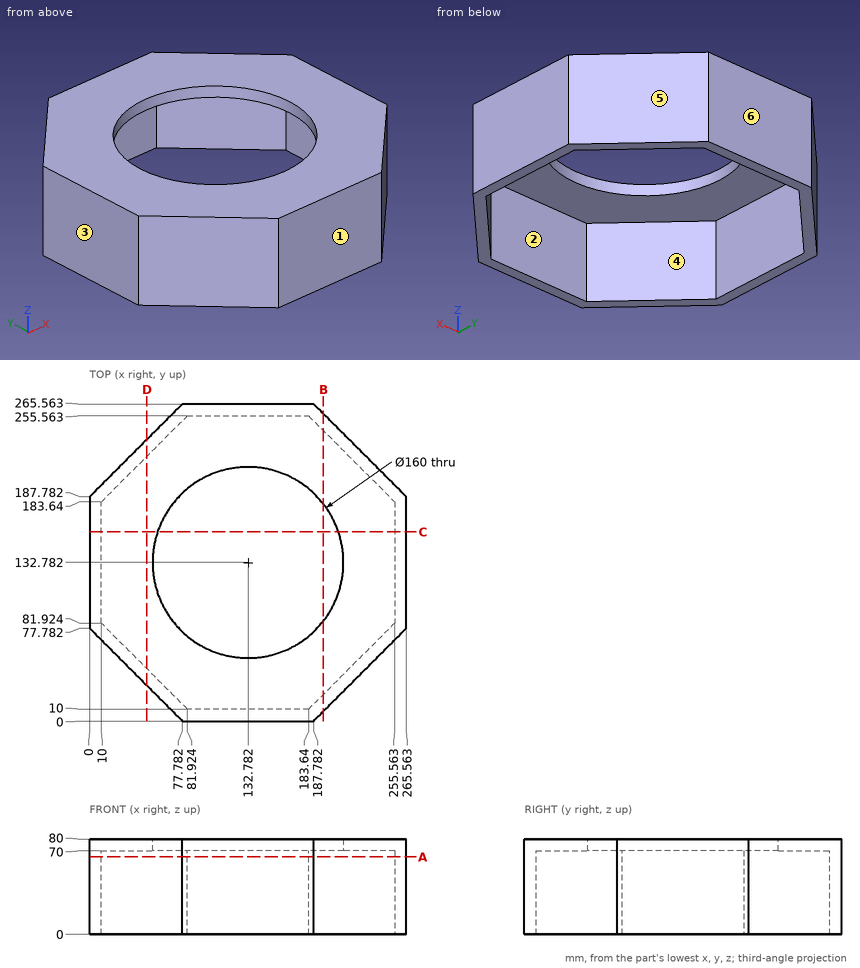
Can you work these out from the drawing? Everything is in mm from the part's minimum corner. A direction names the side the tool comes from. Round coordinates to 2 decimals unless told otherwise and drop trailing zeros. Order: outer loops, then holes, each group sorted by start corner. A loop starts at its lowest first (then second) coordinate and runs counter-clockwise, first axis right, second up. Notation, with made-up numbers: (-27.75, 16.5) - (-18.75, 16.5) arc R9 cw to (-18.75, 23.5) - close; hole circle Ø5 at (3, 31). An arc over 180 degrees is marked (long way). Answer in a Markdown table with one row per item.
(1) Suppose I cut it at A-A, the plane z = 65. Please give me the cut outline in (x, y).
From the geometry:
| item | result |
|---|---|
| outline | (0, 77.78) - (77.78, 0) - (187.78, 0) - (265.56, 77.78) - (265.56, 187.78) - (187.78, 265.56) - (77.78, 265.56) - (0, 187.78) - close; hole (10, 81.92) - (81.92, 10) - (183.64, 10) - (255.56, 81.92) - (255.56, 183.64) - (183.64, 255.56) - (81.92, 255.56) - (10, 183.64) - close |
(2) Suppose I cut it at C-C, the plane y = 158.5. Please give me the cut outline in (x, z) (1 decimal).
From the geometry:
| item | result |
|---|---|
| outline | (0, 0) - (10, 0) - (10, 70) - (57, 70) - (57, 80) - (0, 80) - close; (208.5, 70) - (255.6, 70) - (255.6, 0) - (265.6, 0) - (265.6, 80) - (208.5, 80) - close |
(3) If we mould it in two halves opening along X, with no side actions, what happens to the marked faces 3, 4, 5 and 6? For each: released by +X, released by -X, zero draft, split by the parting line, or undercut.
From the geometry:
| item | result |
|---|---|
| face 3 | released by -X |
| face 4 | undercut |
| face 5 | released by +X |
| face 6 | zero draft |
(4) Please list where these lines run through material, in increasing order: L1, parallel to Y at x = 95.5, z = 49; L2, parallel to Z at x = 69, y = 53. Write a range as from..to.
From the geometry:
| item | result |
|---|---|
| L1 | y = 0..10, 255.56..265.56 |
| L2 | z = 70..80 |
(5) Suppose I cut it at D-D, the plane x = 48. Please give me the cut outline in (y, z), plus the area to 3 significant figures.
From the geometry:
| item | result |
|---|---|
| outline | (29.78, 0) - (43.92, 0) - (43.92, 70) - (221.64, 70) - (221.64, 0) - (235.78, 0) - (235.78, 80) - (29.78, 80) - close |
| area | 4,040 mm2 |
(6) Suppose I cut it at B-B, the plane x = 196. Please give me the cut outline in (y, z) (1 decimal), plus the area to 3 significant figures.
From the geometry:
| item | result |
|---|---|
| outline | (8.2, 0) - (22.4, 0) - (22.4, 70) - (83.8, 70) - (83.8, 80) - (8.2, 80) - close; (181.8, 70) - (243.2, 70) - (243.2, 0) - (257.3, 0) - (257.3, 80) - (181.8, 80) - close |
| area | 3,490 mm2 |
(7) For P1, Ø4, axis at y = 198, z = 62.5, coming from the +X side (1 decimal), with a flat end and sliding along its axis, tell me the tip position at first contact or that it passes through.
From the geometry:
| item | result |
|---|---|
| P1 | stops at x = 257.3 |
(8) Which directions (+Z, -Z, +X, -X, +Y, -Y) give clear straight access to the entire face, cutting with the end or side of a thin tool? Please do the marked faces 1 and 2.
From the geometry:
| item | result |
|---|---|
| face 1 | +Z, -Z, +X, -X, -Y |
| face 2 | -Z |
